from build123d import *

# Parameters (mm, degrees)
EXTRUDE_THIN1_DEPTH = 60
BOSS_EXTRUDE2_DEPTH = 5
SKETCH4_R           = 5.5
BOSS_EXTRUDE3_DEPTH = 25
SKETCH5_R           = 6
BOSS_EXTRUDE4_DEPTH = 25
SKETCH6_R           = 4.372501997
BOSS_EXTRUDE5_DEPTH = 35
CHAMFER1_SIZE       = 1


with BuildPart() as part:
    # Sketch2 → Extrude-Thin1 (new body)
    with BuildSketch(Plane.XY):
        Polygon((0, 0), (0, 25), (25, 25), (25, 23), (2, 23), (2, 0), align=None)
    extrude(amount=EXTRUDE_THIN1_DEPTH)

    # Sketch3 → Boss-Extrude2 (add, symmetric)
    with BuildSketch(Plane(origin=(0, 25, 0), x_dir=(1, 0, 0), z_dir=(0, 1, 0))):
        Polygon((11.684931341, -38.911131142), (20.059731616, -35.594448438), (21.374800275, -26.683317296), (14.315068659, -21.088868858), (5.940268384, -24.405551562), (4.625199725, -33.316682704), align=None)
    extrude(amount=BOSS_EXTRUDE2_DEPTH, both=True)

    # Sketch4 → Boss-Extrude3 (add)
    with BuildSketch(Plane(origin=(0, 20, 0), x_dir=(-1, 0, 0), z_dir=(0, -1, 0))):
        with Locations(Location((-13, -29.319447598, 0), (0, 0, 270))):
            Circle(SKETCH4_R)
    extrude(amount=BOSS_EXTRUDE3_DEPTH)

    # Sketch5 → Boss-Extrude4 (add)
    with BuildSketch(Plane(origin=(0, 30, 0), x_dir=(1, 0, 0), z_dir=(0, 1, 0))):
        with Locations(Location((12.519179725, -29.915081058, 0), (0, 0, 270))):
            Circle(SKETCH5_R)
    extrude(amount=BOSS_EXTRUDE4_DEPTH)

    # Sketch6 → Boss-Extrude5 (add)
    with BuildSketch(Plane(origin=(0, 55, 0), x_dir=(1, 0, 0), z_dir=(0, 1, 0))):
        with Locations(Location((12.519179725, -29.915081058, 0), (0, 0, 270))):
            Circle(SKETCH6_R)
    extrude(amount=BOSS_EXTRUDE5_DEPTH)

    # Chamfer1
    chamfer1_edges = [part.edges().sort_by_distance(p)[0] for p in [
        (13, -5, 23.819447598),
        (12.519179725, 55, 25.542579061),
        (12.519179725, 90, 25.542579061),
    ]]
    chamfer(chamfer1_edges, length=CHAMFER1_SIZE)


solid = part.part
Design review of the part built by this model. Coordinates are the model's own, in mm. A direction names the side the tool comes from. Coordinates: 2 decimals unless noted, no trailing zeros. Order: outer loops, then holes, each group sorted by start corner. A loop starts at its lowest first (then second) coordinate and runs counter-clockwise, first axis right, second up. Notation, with made-up numbers: (78, 7) - (113, 7) arc R27 ccw to (113, 34) - close; hole circle Ø11 at (17, 76). An arc over 180 degrees is marked (long way). Put each result on its own line as item: value.
1) Take a section at A-A, the plane y = 11. Give the boundary of the cut face in (x, z).
Response values:
outline: (0, 0) - (2, 0) - (2, 60) - (0, 60) - close; circle Ø11 at (13, 29.32)
2) Wall thickness on L1, parallel to Y at x = 2.5, z = 55.5; L2, parallel to X at y = 7.5, z = 50.5; L3, parallel to Z at x = 12, y = 36.5: over which ranges is each line inside the solid? List them lowest first. Write a range as from..to.
Response values:
L1: y = 23..25
L2: x = 0..2
L3: z = 23.94..35.89
3) Take a section at B-B, the plane z = 19.5. Give the boundary of the cut face in (x, y).
Response values:
outline: (0, 0) - (2, 0) - (2, 23) - (25, 23) - (25, 25) - (0, 25) - close
4) Insertion check: P1, Ø6, axis at x = 8, z = 7, coming from the -Y side; P2, Ø10, axis at x = 17.5, z = 31, coming from the -Y side; P3, Ø6, axis at x = 4.5, y = 52, coming from the -Z side; P4, Ø6, axis at y = 53.5, z = 25, coming from the +X side. Each pin has a flat end and moves straight along its axis. Give the tip position at first contact, or say it passes through.
Response values:
P1: stops at y = 23
P2: stops at y = -5
P3: stops at z = 26.63
P4: stops at x = 18.21
5) Tool access review of faces 4 (the face through (10.186, 27.535, 22.724)), 5 (the face through (20.71, 27.54, 31.2)), 6 (the face through (9.859, 72.269, 26.445)), 7 (the face through (20.71, 21.52, 31.2)): name each direction out of +Z, -Z, +X, -X, +Y, -Y from which nothing blocks a thin tool from reaching the whole face with its end or side.
Response values:
face 4: -Z, -X, +Y
face 5: +Z, +X, +Y
face 6: +Y
face 7: +Z, +X, -Y
6) Take a section at D-D, the plane y = 83. Give the boundary of the cut face in (x, z) (1 decimal).
Response values:
outline: circle Ø8.7 at (12.5, 29.9)
7) The part is to be moulded in two halves that separate along X. For faces 1 (the face through (5.29, 27.54, 28.8)), 2 (the face through (25, 24, 30)), 3 (the face through (8.106, 21.521, 36.075)), say which applies: released by +X, released by -X, zero draft, split by the parting line, or undercut.
Response values:
face 1: released by -X
face 2: released by +X
face 3: undercut
8) Take a section at C-C, the plane x = 22.5. Give the boundary of the cut face in (y, z).
Response values:
outline: (23, 0) - (25, 0) - (25, 60) - (23, 60) - close
